from build123d import *

# Parameters (mm, degrees)
BOSS_EXTRUDE1_DEPTH   = 10
M4_TAPPED_HOLE1_D     = 3.3
M4_TAPPED_HOLE1_DEPTH = 10.1
M4_TAPPED_HOLE1_TIP   = 0.991420021
M4_TAPPED_HOLE2_D     = 3.3
M4_TAPPED_HOLE2_DEPTH = 10.1
M4_TAPPED_HOLE2_TIP   = 0.991420021


with BuildPart() as part:
    # Sketch1 → Boss-Extrude1 (new body)
    with BuildSketch(Plane(origin=(0, 0, 0), x_dir=(0, 0, -1), z_dir=(1, 0, 0))):
        Polygon((0, 0), (0, 80), (10, 80), (53, 10), (53, 0), align=None)
    extrude(amount=BOSS_EXTRUDE1_DEPTH)

    # M4 Tapped Hole1
    with Locations(Plane.XY):
        with Locations((5, 65), (5, 15)):
            Hole(M4_TAPPED_HOLE1_D / 2, depth=M4_TAPPED_HOLE1_DEPTH)
            with Locations((0, 0, -(M4_TAPPED_HOLE1_DEPTH + M4_TAPPED_HOLE1_TIP / 2))):  # 118° drill point
                Cone(0, M4_TAPPED_HOLE1_D / 2, M4_TAPPED_HOLE1_TIP, mode=Mode.SUBTRACT)

    # M4 Tapped Hole2
    with Locations(Plane(origin=(0, 0, 0), x_dir=(-1, 0, 0), z_dir=(0, -1, 0))):
        with Locations((-5, 43), (-5, 8)):
            Hole(M4_TAPPED_HOLE2_D / 2, depth=M4_TAPPED_HOLE2_DEPTH)
            with Locations((0, 0, -(M4_TAPPED_HOLE2_DEPTH + M4_TAPPED_HOLE2_TIP / 2))):  # 118° drill point
                Cone(0, M4_TAPPED_HOLE2_D / 2, M4_TAPPED_HOLE2_TIP, mode=Mode.SUBTRACT)


solid = part.part
The listing builds one solid part. Answer for the finished solid, in the listing's coordinates (mm). A direction names the side the tool comes from. Give positions to 0.01 mm unless a question says otherwise; leave off trailing zeros. Write each loop counter-clockwise with the first axis right and the second up, starting at its lowest first coordinate (ties: lowest second). Pieces come first, ordered by that corner, then holes. Notation, with made-up numbers: (89.5, 13.25) -> (107.5, 13.25) arc R22 ccw to (107.5, 30.25) -> close; hole circle Ø8 at (12, 0). An arc over 180 degrees is marked (long way). Use a Markdown table: item, result.
(1) For faces 5 (the cylindrical face through (3.784, 5.121, -9.115)), 6 (the flat face through (10, 32, -21)), 7 (the cylindrical face through (6.65, 15.07, -5.12)), determine the directions among +Z, -Z, +X, -X, +Y, -Y from which every point of the face is accessible in a straight line to the end or side of a thin tool.
Return value:
| item | result |
|---|---|
| face 5 | -Y |
| face 6 | +Z, -Z, +X, +Y, -Y |
| face 7 | +Z |
(2) Section C-C, the plane y = 50 is taken. Determine the outline of the cut face in (x, z).
Return value:
| item | result |
|---|---|
| outline | (0, -28.43) -> (10, -28.43) -> (10, 0) -> (0, 0) -> close |
(3) Section B-B, the plane z = -29.5 is taken. Determine the outline of the cut face in (x, y).
Return value:
| item | result |
|---|---|
| outline | (0, 0) -> (10, 0) -> (10, 48.26) -> (0, 48.26) -> close |
(4) Section A-A, the plane x = 9 is taken. Determine the outline of the cut face in (y, z).
Return value:
| item | result |
|---|---|
| outline | (0, -53) -> (10, -53) -> (80, -10) -> (80, 0) -> (0, 0) -> close |
(5) Flat-ended cylindrical pins translate along their axes: P1, Ø1, axis at x = 8.5, z = -11.5, coming from the +Y side; P2, Ø6, axis at y = 18.5, z = -47, coming from the -X side; P3, Ø3, axis at x = 5, y = 15, coming from the +Z side; P4, Ø3, axis at x = 5, z = -8, coming from the -Y side. Find the tip coordinate at first contact, or state that the pin passes through.
Return value:
| item | result |
|---|---|
| P1 | y = 78.37 |
| P2 | x = 0 |
| P3 | z = -10.19 |
| P4 | y = 10.19 |
(6) Find the intervals of material crossed by probe 1 along Y at (x, z) = (5, -4.75); probe 2 along Z at (x, y) = (5, 8); probe 3 along X at (y, z) = (3, -43), in increasing order. Write a range as from..to.
Return value:
| item | result |
|---|---|
| probe 1 | 0..13.35, 16.65..63.35, 66.65..80 |
| probe 2 | -53..-44.65, -41.35..-9.65, -6.35..0 |
| probe 3 | 0..3.35, 6.65..10 |
(7) Determine the mould class of faces 1 (the cylindrical face through (4.785, 5.121, -44.636)), 2 (the flat face through (4.93, 45.49, -31.2)), 3 (the flat face through (0, 32, -21)), 4 (the conical face through (5.04, 10.92, -8.28)) for opening direction X: released by +X, released by -X, zero draft, split by the parting line, or undercut.
Return value:
| item | result |
|---|---|
| face 1 | undercut |
| face 2 | zero draft |
| face 3 | released by -X |
| face 4 | undercut |
